Work out the finished part from the listing and answer in its coordinate system (mm). Face numbers are marked on the shaded views. Coordinates: 2 decimals unless noted, no trailing zeros. Write each loop counter-clockwise with the first axis right and the second up, starting at its lowest first coordinate (ties: lowest second). Pieces come first, ordered by that corner, then holes. Notation, with made-up numbers: (-14.5, 22) - (39.5, 22) arc R29 ccw to (39.5, 61) - close; hole circle Ø4 at (4.5, 32.25). An arc over 180 degrees is marked (long way). Use one line per item in the form item = value. Start each with the question number.
Item 1: A cutting plane is placed at C-C (z = -132.5). Write down the section's boundary in (x, y).
Item 2: Determine the mould class of the marked faces 1, 2, 3 and 4 for opening direction Y: released by +Y, released by -Y, zero draft, split by the parting line, or undercut.
Item 3: Consider probe 1 along X at (y, z) = (49.1, 0); probe 2 along Y at (x, z) = (132, 38.5); probe 3 along X at (y, z) = (22.5, 0). Determine where each line is inside the solid, lowest interval first.
Item 4: A cutting plane is placed at B-B (x = 0). Write down the section's boundary in (y, z).
Item 5: A cutting plane is placed at A-A (z = 0). Write down the section's boundary in (x, y).
Item 6: A cutting plane is placed at D-D (x = -79.5). Write down the section's boundary in (y, z), then the cut area to 3 significant figures.
Item 7: Given pin 1 (4 mm diameter, centred on y = 18.5, z = -92, fed in from +X); pin 2 (2 mm diameter, centred on x = -65.5, y = 5, fed in from -Z); pin 3 (22.5 mm diameter, centred on x = 0, z = 0, fed in from -Y); pin 4 (10 mm diameter, centred on y = 15.5, z = -103.5, fed in from +X), each flat-ended and moving along its own axis, determine where each tip first touches the part or whether it passes through.
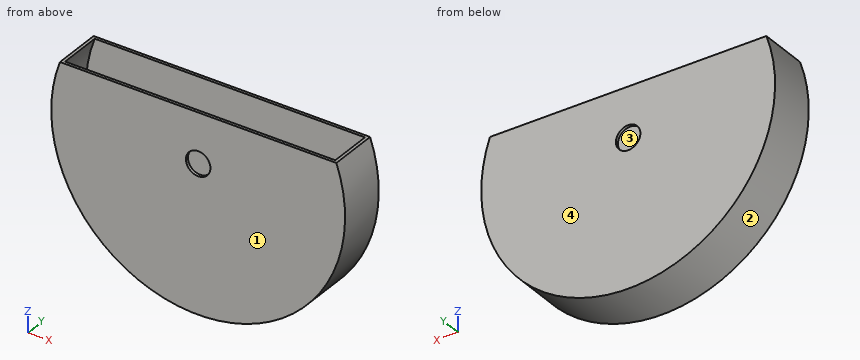
from build123d import *

# Parameters (mm, degrees)
BOSS_EXTRUDE1_DEPTH     = 50
SHELL1_T                = -3
CUT_EXTRUDE1_DEPTH      = 218.944947177
CUT_EXTRUDE1_DEPTH_BACK = 218.944947177
SKETCH2_R               = 12.5


with BuildPart() as part:
    # Sketch1 → Boss-Extrude1 (new body)
    with BuildSketch(Plane(origin=(0, 0, 0), x_dir=(1, 0, 0), z_dir=(0, 1, 0))):
        with BuildLine():
            Line((-141.13085598, -50.814185916), (141.13085598, -50.814185916))
            ThreePointArc((141.13085598, -50.814185916), (0, 150), (-141.13085598, -50.814185916))
        make_face()
    extrude(amount=BOSS_EXTRUDE1_DEPTH)

    # Shell1
    shell1_openings = [part.faces().sort_by_distance(p)[0] for p in [
        (0, 25, 50.814185916),
    ]]
    offset(amount=SHELL1_T, openings=shell1_openings)

    # Sketch2 → Cut-Extrude1 (cut, two sides: drawn at the far end of the back side and taken through both)
    with BuildSketch(Plane(origin=(0, 50, 0), x_dir=(1, 0, 0), z_dir=(0, 1, 0)).offset(-CUT_EXTRUDE1_DEPTH_BACK)):
        with Locations(Location((0, 0, 0), (0, 0, 270))):
            Circle(SKETCH2_R)
    extrude(amount=CUT_EXTRUDE1_DEPTH + CUT_EXTRUDE1_DEPTH_BACK, mode=Mode.SUBTRACT)


solid = part.part
Answer:
q1.outline = (-70.31, 0) - (70.31, 0) - (70.31, 50) - (-70.31, 50) - close; hole (-63.66, 3) - (63.66, 3) - (63.66, 47) - (-63.66, 47) - close
q2.face_1 = released by -Y
q2.face_2 = zero draft
q2.face_3 = undercut
q2.face_4 = released by +Y
q3.probe_1 = -150 to -12.5, 12.5 to 150
q3.probe_2 = 0 to 3, 47 to 50
q3.probe_3 = -150 to -147, 147 to 150
q4.outline = (0, -150) - (50, -150) - (50, -12.5) - (47, -12.5) - (47, -147) - (3, -147) - (3, -12.5) - (0, -12.5) - close; (0, 12.5) - (3, 12.5) - (3, 50.81) - (0, 50.81) - close; (47, 12.5) - (50, 12.5) - (50, 50.81) - (47, 50.81) - close
q5.outline = (-150, 0) - (-12.5, 0) - (-12.5, 3) - (-147, 3) - (-147, 47) - (-12.5, 47) - (-12.5, 50) - (-150, 50) - close; (12.5, 0) - (150, 0) - (150, 50) - (12.5, 50) - (12.5, 47) - (147, 47) - (147, 3) - (12.5, 3) - close
q6.outline = (0, -127.2) - (50, -127.2) - (50, 50.81) - (47, 50.81) - (47, -123.65) - (3, -123.65) - (3, 50.81) - (0, 50.81) - close
q6.area = 1,220 mm²
q7.pin_1 = 120
q7.pin_2 = -135.42
q7.pin_3 = through
q7.pin_4 = 113.13
